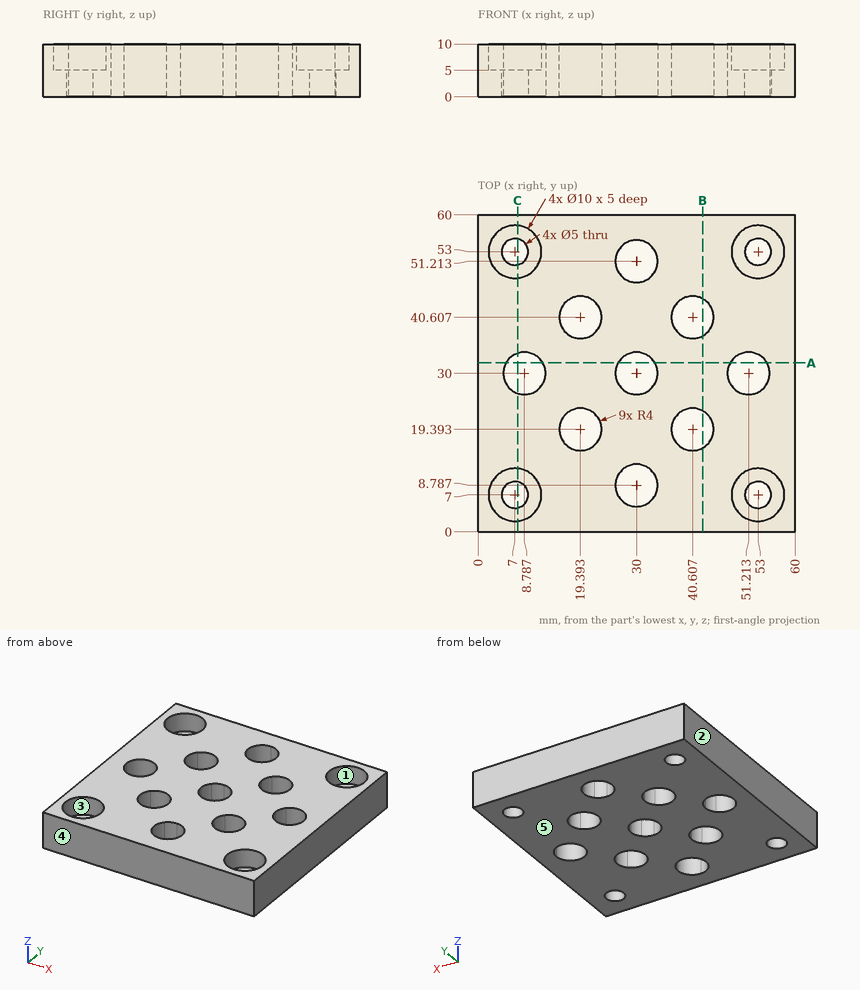
For this review, use the dimensioned drawing (mm, ordinates from the lowest corner) and the shaded views. A direction names the side the tool comes from. Give positions to 0.01 mm unless a question says otherwise; leave off trailing zeros. Write each loop counter-clockwise with the first axis right and the second up, starting at its lowest first coordinate (ties: lowest second). Pieces come first, ordered by that corner, then holes.
(1) Consider section C-C, the plane x = 7.5. Give the number of separate pieces and of enclosed holes in the cut face, and give its area (3 significant figures).
(2) The part is to be moulded in two halves that separate along Y. For the marked faces 3, 4 and 5, say which applies: released by +Y, released by -Y, zero draft, split by the parting line, or undercut.
(3) For P1, Ø4.5, axis at x = 7, y = 53, coming from the -Z side; P2, Ø6, axis at x = 53, y = 7, coming from the -Z side; P3, Ø3, axis at x = 6.5, y = 9, coming from the +Z side, all flat-tipped, find the tip position at first contact; note any pin that passes through.
(4) Consider section A-A, the plane y = 32. Give the boundary of the cut face in (x, z).
(5) Tool access review of the marked faces 1 and 2: name each direction out of +Z, -Z, +X, -X, +Y, -Y from which nothing blocks a thin tool from reaching the whole face with its end or side.
(6) To check wall thickness, follow L1, parallel to Y at x = 19.5, z = 3.5 (1 decimal); L2, parallel to Y at x = 7, z = 2.95; L3, parallel to Y at x = 37.5, z = 0.5 (1 decimal). State the ranges of each line that lie inside material, in increasing order.
(7) Consider section B-B, the plane x = 42.5. Give the boundary of the cut face in (y, z), and give its area (3 significant figures).
Returned:
1. separate pieces: 4
1. enclosed holes: 0
1. area: 376 mm2
2. face 3: undercut
2. face 4: released by -Y
2. face 5: zero draft
3. P1: passes through
3. P2: stops at z = 0
3. P3: stops at z = 5
4. outline: (0, 0) - (5.32, 0) - (5.32, 10) - (0, 10) - close; (12.25, 0) - (26.54, 0) - (26.54, 10) - (12.25, 10) - close; (33.46, 0) - (47.75, 0) - (47.75, 10) - (33.46, 10) - close; (54.68, 0) - (60, 0) - (60, 10) - (54.68, 10) - close
5. face 1: +Z
5. face 2: +Z, -Z, -X, +Y, -Y
6. L1: y = 0 to 15.4, 23.4 to 36.6, 44.6 to 60
6. L2: y = 0 to 4.5, 9.5 to 26.42, 33.58 to 50.5, 55.5 to 60
6. L3: y = 0 to 16.9, 21.9 to 38.1, 43.1 to 60
7. outline: (0, 0) - (15.87, 0) - (15.87, 10) - (0, 10) - close; (22.92, 0) - (37.08, 0) - (37.08, 10) - (22.92, 10) - close; (44.13, 0) - (60, 0) - (60, 10) - (44.13, 10) - close
7. area: 459 mm2
